Part model, mm, in its own coordinate system. A direction names the side the tool comes from. Round coordinates to 2 decimals unless told otherwise and drop trailing zeros. Loops run counter-clockwise (first coordinate to the right, second up) from the corner with the lowest first, then second, coordinate; pieces in that order, holes last. Notation, with made-up numbers: M -20,-21 L -6,-21 A8 cw -6,-8 Z; hole C 54,85 d4. An arc over 180 degrees is marked long. Put each result on its own line as item: value. Start each with the question number.
```python
from build123d import *

# Parameters (mm, degrees)
FLANGE_DISC_SKETCH_R          = 80
FLANGE_DISC_160_DEPTH         = 11
HUB_SKETCH_R                  = 40
HUB_SKETCH_R_2                = 30
HUB_80X_60_DEPTH              = 28
ROUND_BOSS_SKETCH_R           = 30
ROUND_BOSS_15MM_DEPTH         = 15
MOUNTING_LUG_SKETCH_R         = 7
MOUNTING_LUG_DEPTH            = 24
MOUNTING_LUG_PATTERN_4X_COUNT = 4
RIM_START                     = -24
RIM_SLOT_CUT_DEPTH            = 24
RIM_SLOT_PATTERN_4X_COUNT     = 4


with BuildPart() as part:
    # Flange Disc Sketch → Flange Disc Ø160 (new body)
    with BuildSketch(Plane.XY):
        Circle(FLANGE_DISC_SKETCH_R)
    extrude(amount=FLANGE_DISC_160_DEPTH)

    # Hub Sketch → Hub Ø80xØ60 (add)
    with BuildSketch(Plane.XY.offset(11)):
        Circle(HUB_SKETCH_R)
        Circle(HUB_SKETCH_R_2, mode=Mode.SUBTRACT)
    extrude(amount=HUB_80X_60_DEPTH)

    # Round Boss Sketch → Round Boss 15mm (add)
    with BuildSketch(Plane.XY.offset(11)):
        Circle(ROUND_BOSS_SKETCH_R)
    extrude(amount=ROUND_BOSS_15MM_DEPTH)

    # Mounting Lug Sketch → Mounting Lug (add)
    with BuildSketch(Plane.XY.offset(11)):
        with BuildLine():
            Line((16.595787662, 36.394777536), (28.991378029, 48.790367902))
            ThreePointArc((28.991378029, 48.790367902), (48.790367902, 48.790367902), (48.790367902, 28.991378029))
            Line((48.790367902, 28.991378029), (36.394777536, 16.595787662))
            ThreePointArc((36.394777536, 16.595787662), (28.284271247, 28.284271247), (16.595787662, 36.394777536))
        make_face()
        with Locations((38.890872965, 38.890872965)):
            Circle(MOUNTING_LUG_SKETCH_R, mode=Mode.SUBTRACT)
    mounting_lug = extrude(amount=MOUNTING_LUG_DEPTH)

    # Mounting Lug Pattern 4x: Mounting Lug ×4 about axis
    mounting_lug_pattern_4x_axis = Axis((0, 0, 0), (0, 0, 1))
    for i in range(1, MOUNTING_LUG_PATTERN_4X_COUNT):
        add(mounting_lug.rotate(mounting_lug_pattern_4x_axis, i * 360 / MOUNTING_LUG_PATTERN_4X_COUNT))

    # Rim Slot Sketch → Rim Slot Cut (cut)
    with BuildSketch(Plane.XY.offset(11).offset(RIM_START)):
        with BuildLine():
            Line((62.5, 8), (79.598994969, 8))
            ThreePointArc((79.598994969, 8), (80, 0), (79.598994969, -8))
            Line((79.598994969, -8), (62.5, -8))
            ThreePointArc((62.5, -8), (54.5, 0), (62.5, 8))
        make_face()
    rim_slot_cut = extrude(amount=RIM_SLOT_CUT_DEPTH, mode=Mode.SUBTRACT)

    # Rim Slot Pattern 4x: Rim Slot Cut ×4 about axis
    rim_slot_pattern_4x_axis = Axis((0, 0, 0), (0, 0, 1))
    for i in range(1, RIM_SLOT_PATTERN_4X_COUNT):
        add(rim_slot_cut.rotate(rim_slot_pattern_4x_axis, i * 360 / RIM_SLOT_PATTERN_4X_COUNT), mode=Mode.SUBTRACT)


solid = part.part
```
1. Cut at A-A, the plane x = 0. Give the cut face in (y, z).
2. Drop flat-ended pins along their axis: pin 1 (18 mm diameter, centred on x = -39, y = 41.5, fed in from +Z); pin 2 (10 mm diameter, centred on x = 59.5, y = -22.5, fed in from +Z); pin 3 (8 mm diameter, centred on y = 31, z = 33.5, fed in from -X); pin 4 (12.5 mm diameter, centred on x = 38.89, y = -38.89, fed in from -Z). Give the stop position or say it passes through.
3. Cut at B-B, the plane z = 19.5. Give the cut face in (x, y).
4. Which spindle directions (+Z, -Z, +X, -X, +Y, -Y) get a long thin tool onto all of the face, cutting with end or side? Do faces 4 (the flat face through (39, -39, 11)), 5 (the flat face through (71, -8, 5)), 6 (the flat face through (-42.5, 22.7, 22.8)), 7 (the flat face through (31, 39, 35)), 8 (the flat face through (-71, -8, 5)). Say none if no direction does.
5. Mould opens along Y. For faces 1 (the cylindrical face through (56.02, -57.11, 5.42)), 2 (the flat face through (39, 39, 11)), 3 (the flat face through (39, -31, 35)) say: released by +Y, released by -Y, zero draft, split by the parting line, or undercut.
6. Wall check: L1, parallel to Y at x = 0, z = 33.5; L2, parallel to Y at x = 45, z = 21; L3, parallel to Z at x = -58.5, y = -27.5. Give the ranges that are in metal, low to high.
7. Cut at D-D, the plane y = 65.5. Give the cut face in (x, z), and give its area (3 significant figures).
Results list:
1. outline: M -54.5,0 L 54.5,0 L 54.5,11 L 40,11 L 40,39 L 30,39 L 30,26 L -30,26 L -30,39 L -40,39 L -40,11 L -54.5,11 Z
2. pin 1: stops at z = 35
2. pin 2: stops at z = 11
2. pin 3: stops at x = -52.34
2. pin 4: stops at z = 0
3. outline: M -48.79,-28.99 A14 ccw -28.99,-48.79 L -16.6,-36.39 A40 ccw 16.6,-36.39 L 28.99,-48.79 A14 ccw 48.79,-28.99 L 36.39,-16.6 A40 ccw 36.39,16.6 L 48.79,28.99 A14 ccw 28.99,48.79 L 16.6,36.39 A40 ccw -16.6,36.39 L -28.99,48.79 A14 ccw -48.79,28.99 L -36.39,16.6 A40 ccw -36.39,-16.6 Z; hole C -38.89,-38.89 d14; hole C -38.89,38.89 d14; hole C 38.89,-38.89 d14; hole C 38.89,38.89 d14
4. face 4: +Z
4. face 5: +Z, -Z, +X
4. face 6: +Z, -X
4. face 7: +Z, +X, +Y
4. face 8: +Z, -Z, -X
5. face 1: released by -Y
5. face 2: undercut
5. face 3: zero draft
6. L1: y = -40 to -30, 30 to 40
6. L2: y = -51.49 to -42.31, -35.47 to -25.2, 25.2 to 35.47, 42.31 to 51.49
6. L3: z = 0 to 11
7. outline: M -45.93,0 L -8,0 L -8,11 L -45.93,11 Z; M 8,0 L 45.93,0 L 45.93,11 L 8,11 Z
7. area: 835 mm^2
